```python
from build123d import *

# Parameters (mm, degrees)
EXTRUDE_1_DEPTH     = 40
SKETCH_2_R          = 16.5
CUT_EXTRUDE_1_DEPTH = 2


with BuildPart() as part:
    # 草图1 → 凸台-拉伸1 (new body)
    with BuildSketch(Plane(origin=(0, 0, 0), x_dir=(1, 0, 0), z_dir=(0, 1, 0))):
        Polygon((0, 0), (40, 0), (40, -39), (34, -39), (0, -7), align=None)
    extrude(amount=EXTRUDE_1_DEPTH)

    # 草图2 → 切除-拉伸1 (cut)
    with BuildSketch(Plane(origin=(40, 0, 0), x_dir=(0, 0, -1), z_dir=(1, 0, 0))):
        with Locations((-19.5, 20)):
            Circle(SKETCH_2_R)
    extrude(amount=-CUT_EXTRUDE_1_DEPTH, mode=Mode.SUBTRACT)


solid = part.part
```
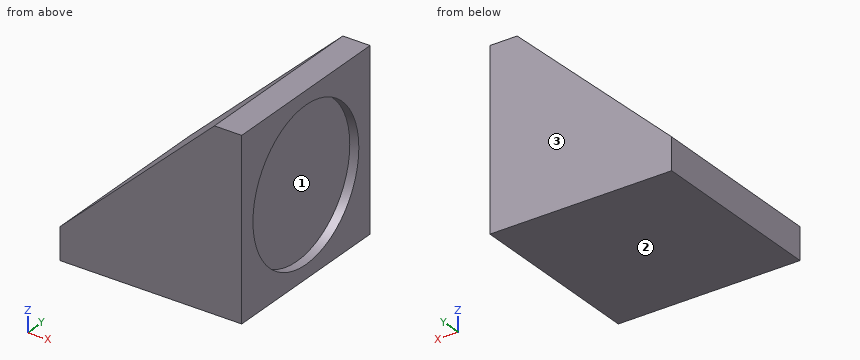
CAD build for the part. Positions are in the model's coordinates, mm. Face numbers are marked on the shaded views. Give positions to 0.01 mm unless a question says otherwise; leave off trailing zeros. Loops run counter-clockwise (first coordinate to the right, second up) from the corner with the lowest first, then second, coordinate; pieces in that order, holes last. Notation, with made-up numbers: (68.5, -19.75) - (79.5, -19.75) arc R21 ccw to (79.5, 5.25) - close; hole circle Ø10 at (38, 51.25). An arc over 180 degrees is marked (long way). Put each result on its own line as item: value.
Q1. Slice it at C-C (x = 27). Give the cut face in (y, z).
Filled in:
outline: (0, 0) - (40, 0) - (40, 32.41) - (0, 32.41) - close
Q2. Probe line 1 along Y through (x, z) = (38.95, 19.5); line 2 along X through (y, z) = (6, 34.5); line 3 along X through (y, z) = (7.5, 17) (3 decimals). List the from-to ranges inside material, lowest first.
Filled in:
line 1: y = 0 to 3.5, 36.5 to 40
line 2: x = 29.22 to 40
line 3: x = 10.625 to 38
Q3. Slice it at B-B (z = 13.5). Give the cut face in (x, y).
Filled in:
outline: (6.91, 0) - (40, 0) - (40, 4.63) - (38, 4.63) - (38, 35.37) - (40, 35.37) - (40, 40) - (6.91, 40) - close
Q4. Slice it at A-A (y = 20). Give the cut face in (x, z).
Filled in:
outline: (0, 0) - (40, 0) - (40, 3) - (38, 3) - (38, 36) - (40, 36) - (40, 39) - (34, 39) - (0, 7) - close
Q5. Slice it at D-D (z = 26). Give the cut face in (x, y), plus the area to 3 significant figures.
Filled in:
outline: (20.19, 0) - (40, 0) - (40, 4.83) - (38, 4.83) - (38, 35.17) - (40, 35.17) - (40, 40) - (20.19, 40) - close
area: 732 mm²
Q6. Mould opens along Z. For the marked faces 1, 2 and 3 say: pulls with the +Z half, pulls with the -Z half, needs draft (parallel to the pull), parting line crosses it, or undercut.
Filled in:
face 1: undercut
face 2: pulls with the -Z half
face 3: needs draft
Q7. Flat gauge pins, fed straight in: pin 1 (5 mm diameter, centred on y = 24, z = 23, fed in from -X); pin 2 (2 mm diameter, centred on y = 10.5, z = 29.5, fed in from +X). Where does each tip first touch, or does it go through?
Filled in:
pin 1: stops at x = 14.34
pin 2: stops at x = 38
